```python
from build123d import *

# Parameters (mm, degrees)
SKETCH1_R           = 5
BOSS_EXTRUDE1_DEPTH = 390
SKETCH2_W           = 10
SKETCH2_H           = 15
BOSS_EXTRUDE2_DEPTH = 20
SKETCH3_W           = 10
SKETCH3_H           = 15
BOSS_EXTRUDE3_DEPTH = 20
SKETCH4_R           = 5
CUT_EXTRUDE1_DEPTH  = 411.190504522


with BuildPart() as part:
    # Sketch1 → Boss-Extrude1 (new body)
    with BuildSketch(Plane.XY):
        Circle(SKETCH1_R)
    extrude(amount=BOSS_EXTRUDE1_DEPTH)

    # Sketch2 → Boss-Extrude2 (add)
    with BuildSketch(Plane(origin=(0, 0, 0), x_dir=(-1, 0, 0), z_dir=(0, 0, -1))):
        Rectangle(SKETCH2_W, SKETCH2_H)
    extrude(amount=BOSS_EXTRUDE2_DEPTH)

    # Sketch3 → Boss-Extrude3 (add)
    with BuildSketch(Plane.XY.offset(390)):
        Rectangle(SKETCH3_W, SKETCH3_H)
    extrude(amount=BOSS_EXTRUDE3_DEPTH)

    # Sketch4 → Cut-Extrude1 (cut, through all)
    with BuildSketch(Plane(origin=(5, 0, 0), x_dir=(0, 0, -1), z_dir=(1, 0, 0))):
        with Locations((12.5, 0)):
            Circle(SKETCH4_R)
        with Locations((-402.5, 0)):
            Circle(SKETCH4_R)
        with BuildLine():
            Line((12.5, -7.5), (27.957175819, -19.344646022))
            Line((27.957175819, -19.344646022), (25.412525065, 11.111642689))
            Line((25.412525065, 11.111642689), (12.5, 7.5))
            ThreePointArc((12.5, 7.5), (20, 0), (12.5, -7.5))
        make_face()
        with BuildLine():
            Line((-402.5, 7.5), (-436.593003508, 16.998965127))
            Line((-436.593003508, 16.998965127), (-417.537871644, -29.426265233))
            Line((-417.537871644, -29.426265233), (-402.5, -7.5))
            ThreePointArc((-402.5, -7.5), (-410, 0), (-402.5, 7.5))
        make_face()
    extrude(amount=-CUT_EXTRUDE1_DEPTH, mode=Mode.SUBTRACT)


solid = part.part
```
CAD build for the part. Positions are in the model's coordinates, mm. A direction names the side the tool comes from. Give positions to 0.01 mm unless a question says otherwise; leave off trailing zeros. Order: outer loops, then holes, each group sorted by start corner. A loop starts at its lowest first (then second) coordinate and runs counter-clockwise, first axis right, second up.
(1) Saw through at A-A, the plane x = -1.5. Give the cut face in (y, z).
(2) Drill centre lines: L1, parallel to Y at x = 0.5, z = 402.5; L2, parallel to Z at x = 3.75, y = 2.5; L3, parallel to Z at x = -1, y = 5.5. Where is each one in solid material? Low to high.
(3) Tool access for faces 1 (the flat face through (-0.1, 5.5, 390)), 2 (the cylindrical face through (-1.08, -4.88, 192.27)), 3 (the flat face through (-0.1, -5.4, 390)), 4 (the cylindrical face through (0, 0, 410)): list every direction of +Z, -Z, +X, -X, +Y, -Y with a clear straight run to the whole face (end or side of a thin tool).
(4) Saw through at B-B, the plane z = 298.5. Give the cut face in (x, y), then the cut area to 3 significant figures.
(5) Flat gauge pins, fed straight in: pin 1 (2 mm diameter, centred on x = -1, y = 4, fed in from +Z); pin 2 (4 mm diameter, centred on x = 0.5, y = -2.5, fed in from -Z); pin 3 (4 mm diameter, centred on x = -1.5, z = 242.5, fed in from -Y). Where does each tip first touch, or does it go through?
(6) Mould opens along Y. For faces 5 (the cylindrical face through (0.07, 1.5, 397.73)), 6 (the flat face through (-5, -1.8, 397.6)), 7 (the cylindrical face through (0.07, 1.5, -17.27)), 8 (the flat face through (0, -7.5, -6)) say: released by +Y, released by -Y, zero draft, split by the parting line, or undercut.
Results found:
1. outline: (-7.5, -12.5) arc R7.5 ccw to (7.5, -12.5) - (7.5, 0) - (4.77, 0) - (4.77, 390) - (7.5, 390) - (7.5, 402.5) arc R7.5 ccw to (-7.5, 402.5) - (-7.5, 390) - (-4.77, 390) - (-4.77, 0) - (-7.5, 0) - close; hole circle Ø10 at (0, -12.5); hole circle Ø10 at (0, 402.5)
2. L1: y = -7.5 to -5, 5 to 7.5
2. L2: z = -19.57 to -16.83, -8.17 to 398.17, 406.83 to 409.57
2. L3: z = -17.6 to 0, 390 to 407.6
3. face 1: +Y
3. face 2: none
3. face 3: -Y
3. face 4: +Z, +X, -X
4. outline: circle Ø10 at (0, 0)
4. area: 78.5 mm2
5. pin 1: stops at z = 409.37
5. pin 2: stops at z = -19.98
5. pin 3: stops at y = -5
6. face 5: undercut
6. face 6: zero draft
6. face 7: undercut
6. face 8: released by -Y
